```python
from build123d import *

# Parameters (mm, degrees)
BASE_PLATE_DEPTH           = 18
MOUNTING_HOLES_SKETCH_R    = 7.5
MOUNTING_HOLES_4X_15_DEPTH = 18
CLEVIS_BASE_BOSS_DEPTH     = 15
CLEVIS_BODY_SKETCH_W       = 10
CLEVIS_BODY_SKETCH_H       = 41
CLEVIS_BODY_DEPTH          = 48
EYE_SPACER_SKETCH_W        = 41
EYE_SPACER_SKETCH_H        = 48
EYE_SPACER_DEPTH           = 5
EYE_LUG_SKETCH_W           = 20
EYE_LUG_SKETCH_H           = 48
EYE_LUG_DEPTH              = 15
EYE_START                  = -15
EYE_LUG_ROUND_END_DEPTH    = 15
EYE_BORE_SKETCH_R          = 12
EYE_BORE_24_DEPTH          = 55
GUSSET_DEPTH               = 48
GUSSET_TRIM_A_DEPTH        = 19
GUSSET_TRIM_B_DEPTH        = 19


with BuildPart() as part:
    # Base Plate Sketch → Base Plate (new body)
    with BuildSketch(Plane.XY):
        with BuildLine():
            Line((15, 0), (90, 0))
            ThreePointArc((90, 0), (100.606601718, 4.393398282), (105, 15))
            Line((105, 15), (105, 83))
            ThreePointArc((105, 83), (100.606601718, 93.606601718), (90, 98))
            Line((90, 98), (15, 98))
            ThreePointArc((15, 98), (4.393398282, 93.606601718), (0, 83))
            Line((0, 83), (0, 15))
            ThreePointArc((0, 15), (4.393398282, 4.393398282), (15, 0))
        make_face()
    extrude(amount=BASE_PLATE_DEPTH)

    # Mounting Holes Sketch → Mounting Holes 4xØ15 (cut)
    with BuildSketch(Plane.XY.offset(18)):
        with Locations((15, 83)):
            Circle(MOUNTING_HOLES_SKETCH_R)
        with Locations((90, 83)):
            Circle(MOUNTING_HOLES_SKETCH_R)
        with Locations((90, 15)):
            Circle(MOUNTING_HOLES_SKETCH_R)
        with Locations((15, 15)):
            Circle(MOUNTING_HOLES_SKETCH_R)
    extrude(amount=-MOUNTING_HOLES_4X_15_DEPTH, mode=Mode.SUBTRACT)

    # Clevis Base Boss Sketch → Clevis Base Boss (add)
    with BuildSketch(Plane.XY.offset(18)):
        with BuildLine():
            Line((80, 73), (45, 73))
            Line((45, 73), (45, 25))
            Line((45, 25), (80, 25))
            ThreePointArc((80, 25), (104, 49), (80, 73))
        make_face()
    extrude(amount=CLEVIS_BASE_BOSS_DEPTH)

    # Clevis Body Sketch → Clevis Body (add)
    with BuildSketch(Plane.XZ.offset(-25)):
        with Locations((50, 53.5)):
            Rectangle(CLEVIS_BODY_SKETCH_W, CLEVIS_BODY_SKETCH_H)
    extrude(amount=-CLEVIS_BODY_DEPTH)

    # Eye Spacer Sketch → Eye Spacer (add)
    with BuildSketch(Plane(origin=(55, 0, 0), x_dir=(0, 0, -1), z_dir=(1, 0, 0))):
        with Locations((-53.5, 49)):
            Rectangle(EYE_SPACER_SKETCH_W, EYE_SPACER_SKETCH_H)
    extrude(amount=EYE_SPACER_DEPTH)

    # Eye Lug Sketch → Eye Lug (add)
    with BuildSketch(Plane.XY.offset(74)):
        with Locations((70, 49)):
            Rectangle(EYE_LUG_SKETCH_W, EYE_LUG_SKETCH_H)
    extrude(amount=-EYE_LUG_DEPTH)

    # Eye Lug Round End Sketch → Eye Lug Round End (add)
    with BuildSketch(Plane.XY.offset(74).offset(EYE_START)):
        with BuildLine():
            Line((80, 73), (80, 25))
            ThreePointArc((80, 25), (104, 49), (80, 73))
        make_face()
    extrude(amount=EYE_LUG_ROUND_END_DEPTH)

    # Eye Bore Sketch → Eye Bore Ø24 (cut)
    with BuildSketch(Plane.XY.offset(74)):
        with Locations((80, 49)):
            Circle(EYE_BORE_SKETCH_R)
    extrude(amount=-EYE_BORE_24_DEPTH, mode=Mode.SUBTRACT)

    # Gusset Sketch → Gusset (add)
    with BuildSketch(Plane.XZ.offset(-25)):
        Polygon((45, 74), (45, 18), (0, 18), align=None)
    extrude(amount=-GUSSET_DEPTH)

    # Gusset Trim A Sketch → Gusset Trim A (cut)
    with BuildSketch(Plane.XZ.offset(-25)):
        Polygon((45, 74), (45, 18), (0, 18), align=None)
    extrude(amount=-GUSSET_TRIM_A_DEPTH, mode=Mode.SUBTRACT)

    # Gusset Trim B Sketch → Gusset Trim B (cut)
    with BuildSketch(Plane(origin=(0, 73, 0), x_dir=(1, 0, 0), z_dir=(0, 1, 0))):
        Polygon((45, -74), (45, -18), (0, -18), align=None)
    extrude(amount=-GUSSET_TRIM_B_DEPTH, mode=Mode.SUBTRACT)


solid = part.part
```
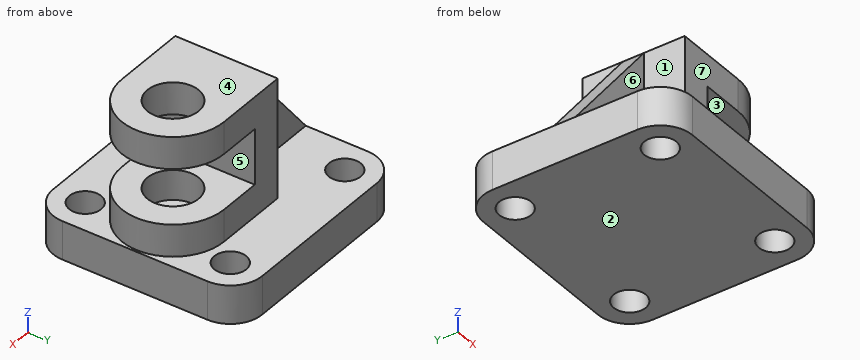
Can you work these out from the model? Positions are in its coordinate system, mm. Face numbers are marked on the shaded views. A direction names the side the tool comes from. Give positions to 0.01 mm unless a question says otherwise; leave off trailing zeros. Order: outer loops, then holes, each group sorted by start corner. A loop starts at its lowest first (then second) coordinate and runs counter-clockwise, first axis right, second up. Notation, with made-up numbers: M 20,56 L 73,56 A15 ccw 73,60 Z; hole C 33,29.25 d6. An arc over 180 degrees is marked long. Write item = value, one per line. Start each with the question number.
Q1. Suppose I cut it at C-C (y = 80). Write out the boundary of the cut face in (x, z), plus the area to 3 significant figures.
Q2. Suppose I cut it at B-B (z = 15). Write out the boundary of the cut face in (x, y), plus the area to 3 significant figures.
Q3. Suppose I cut it at D-D (x = 85). Write out the boundary of the cut face in (y, z), plus the area to 3 significant figures.
Q4. I need wall thicknesses on probe 1 along Y at (x, z) = (15, 4.75); probe 2 along Z at (x, y) = (63, 49.5); probe 3 along Y at (x, z) = (80, 30). Which ranges of each line are inside material? Lowest first, please. Write a range as [from, to].
Q5. We'd pull the mould along Z, two halves only. Please class the marked faces 1, 2, 3 and 4: pulls with the +Z half, pulls with the -Z half, needs draft (parallel to the pull), parting line crosses it, or undercut.
Q6. Will these pins go through, and if not, where does the flat tip stop? pin 1 Ø21 at (y, z) = (39, 43) entering from -X; pin 2 Ø13.5 at (x, z) = (15.5, 40) entering from -Y; pin 3 Ø13.5 at (x, y) = (15, 15) entering from -Z; pin 4 Ø17.5 at (x, z) = (62, 53) entering from +Y.
Q7. Suppose I cut it at A-A (y = 49). Write out the boundary of the cut face in (x, z).
Q8. For the marked faces 5, 6 and 7, which set-ups out of +Z, -Z, +X, -X, +Y, -Y let a thin tool reach every point of the face, with its end or its side?
Check result:
q1.outline = M 0,0 L 8.13,0 L 8.13,18 L 0,18 Z; M 21.87,0 L 83.13,0 L 83.13,18 L 21.87,18 Z; M 96.87,0 L 105,0 L 105,18 L 96.87,18 Z
q1.area = 1,400 mm2
q2.outline = M 0,15 A15 ccw 15,0 L 90,0 A15 ccw 105,15 L 105,83 A15 ccw 90,98 L 15,98 A15 ccw 0,83 Z; hole C 15,15 d15; hole C 15,83 d15; hole C 90,15 d15; hole C 90,83 d15
q2.area = 9,390 mm2
q3.outline = M 0,0 L 9.41,0 L 9.41,18 L 0,18 Z; M 20.59,0 L 77.41,0 L 77.41,18 L 72.47,18 L 72.47,33 L 59.91,33 L 59.91,19 L 38.09,19 L 38.09,33 L 25.53,33 L 25.53,18 L 20.59,18 Z; M 25.53,59 L 38.09,59 L 38.09,74 L 25.53,74 Z; M 59.91,59 L 72.47,59 L 72.47,74 L 59.91,74 Z; M 88.59,0 L 98,0 L 98,18 L 88.59,18 Z
q3.area = 2,140 mm2
q4.probe_1 = [0, 7.5], [22.5, 75.5], [90.5, 98]
q4.probe_2 = [0, 33], [59, 74]
q4.probe_3 = [25, 37], [61, 73]
q5.face_1 = needs draft
q5.face_2 = pulls with the -Z half
q5.face_3 = undercut
q5.face_4 = pulls with the +Z half
q6.pin_1 = 12.67
q6.pin_2 = 44
q6.pin_3 = through
q6.pin_4 = 73
q7.outline = M 0,0 L 105,0 L 105,18 L 104,18 L 104,33 L 92,33 L 92,19 L 68,19 L 68,33 L 60,33 L 60,59 L 68,59 L 68,74 L 45,74 L 0,18 Z; M 92,59 L 104,59 L 104,74 L 92,74 Z
q8.face_5 = +X, +Y, -Y
q8.face_6 = +Z, -X, -Y
q8.face_7 = +Z, +X, -X, -Y
